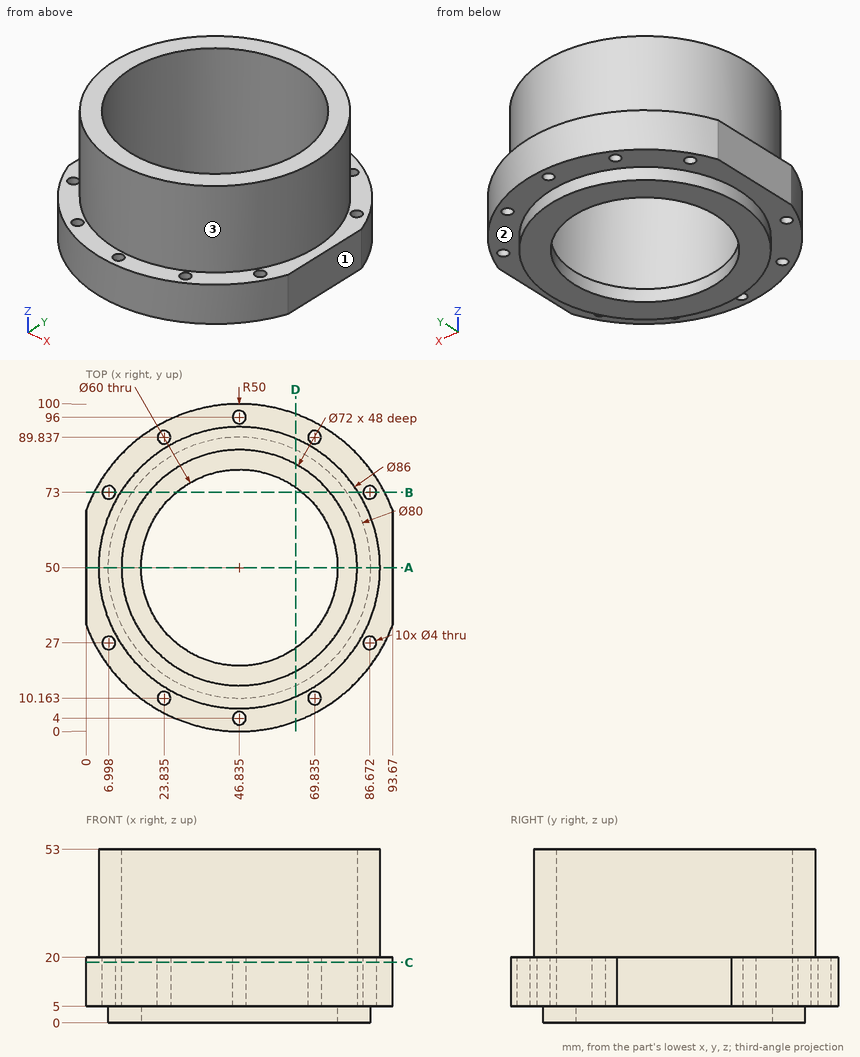
Geometry: see drawing. Coordinates: mm, zero at the bounding-box minimum. A direction names the side the tool comes from. Round coordinates to 2 decimals unless told otherwise and drop trailing zeros. Loops run counter-clockwise (first coordinate to the right, second up) from the corner with the lowest first, then second, coordinate; pieces in that order, holes last. Notation, with made-up numbers: M 3.5,-20.75 L 53.5,-20.75 A19 cw 53.5,-2.75 Z; hole C 56.5,9.5 d4. An arc over 180 degrees is marked long. Use a Markdown table: item, result. Add a question column.
1. Set-up query: the marked faces 1, 2 and 3. Return all of +Z, -Z, +X, -X, +Y, -Y with unobstructed straight access to the full face (end or side cutting, diameter ignored); none if empty.
2. Ray query, line 1 along X through (y, z) = (49, 44.5); line 2 along Z through (x, y) = (77, 68); line 3 along X through (y, z) = (68, 32.5). Return the intervals inside material, ascending. Write a range as [from, to].
3. Cut plane C-C, the plane z = 18.5. State how many separate pieces and enclosed holes the cut face has, and give its area (3 significant figures).
4. Contact query for flat-ended pins moving along their axis: pin 1 (3.5 mm diameter, centred on x = 86.67, y = 73, fed in from +Z); pin 2 (1 mm diameter, centred on x = 80, y = 60, fed in from +Z); pin 3 (5 mm diameter, centred on x = 59, z = 37.5, fed in from -Y); pin 4 (12 mm diameter, centred on x = 60.5, z = 12.5, fed in from +Y). Output: stop coordinate, or through.
5. Cut plane D-D, the plane x = 64. Output: boundary loops of the cut face in (y, z), and give its area (3 significant figures).
6. Cut plane A-A, the plane y = 50. Output: boundary loops of the cut face in (x, z) (3 decimals), and give its area (3 significant figures).
7. Cut plane B-B, the plane y = 73. Output: boundary loops of the cut face in (x, z).
Solution:
| question | item | result |
|---|---|---|
| 1 | face 1 | +Z, -Z, +X, +Y, -Y |
| 1 | face 2 | -Z |
| 1 | face 3 | +Z |
| 2 | line 1 | x = [3.85, 10.85], [82.82, 89.82] |
| 2 | line 2 | z = [0, 5] |
| 2 | line 3 | x = [7.78, 15.66], [78.01, 85.89] |
| 3 | separate pieces | 1 |
| 3 | enclosed holes | 11 |
| 3 | area | 3,510 mm2 |
| 4 | pin 1 | passes through |
| 4 | pin 2 | stops at z = 5 |
| 4 | pin 3 | stops at y = 8.1 |
| 4 | pin 4 | stops at y = 99.41 |
| 5 | outline | M 3.04,5 L 13.87,5 L 13.87,0 L 25.4,0 L 25.4,5 L 18.36,5 L 18.36,53 L 10.57,53 L 10.57,20 L 3.04,20 Z; M 74.6,0 L 86.13,0 L 86.13,5 L 96.96,5 L 96.96,20 L 89.43,20 L 89.43,53 L 81.64,53 L 81.64,5 L 74.6,5 Z |
| 5 | area | 1,090 mm2 |
| 6 | outline | M 0,5 L 6.835,5 L 6.835,0 L 16.835,0 L 16.835,5 L 10.835,5 L 10.835,53 L 3.835,53 L 3.835,20 L 0,20 Z; M 76.835,0 L 86.835,0 L 86.835,5 L 93.67,5 L 93.67,20 L 89.835,20 L 89.835,53 L 82.835,53 L 82.835,5 L 76.835,5 Z |
| 6 | area | 887 mm2 |
| 7 | outline | M 2.44,5 L 5,5 L 5,20 L 2.44,20 Z; M 9,5 L 14.11,5 L 14.11,0 L 27.57,0 L 27.57,5 L 19.14,5 L 19.14,53 L 10.5,53 L 10.5,20 L 9,20 Z; M 66.1,0 L 79.56,0 L 79.56,5 L 84.67,5 L 84.67,20 L 83.17,20 L 83.17,53 L 74.53,53 L 74.53,5 L 66.1,5 Z; M 88.67,5 L 91.23,5 L 91.23,20 L 88.67,20 Z |
